```python
from build123d import *

# Parameters (mm, degrees)
SKETCH1_R           = 11.5
BOSS_EXTRUDE1_DEPTH = 4
SKETCH2_R           = 7.5
BOSS_EXTRUDE2_DEPTH = 42
CHAMFER1_SIZE       = 1
CHAMFER2_SIZE       = 0.5


with BuildPart() as part:
    # Sketch1 → Boss-Extrude1 (new body)
    with BuildSketch(Plane(origin=(0, 0, 0), x_dir=(1, 0, 0), z_dir=(0, 1, 0))):
        with Locations(Location((0, 0, 0), (0, 0, 270))):
            Circle(SKETCH1_R)
    extrude(amount=BOSS_EXTRUDE1_DEPTH)

    # Sketch2 → Boss-Extrude2 (add)
    with BuildSketch(Plane(origin=(0, 4, 0), x_dir=(1, 0, 0), z_dir=(0, 1, 0))):
        with Locations(Location((0, 0, 0), (0, 0, 90))):
            Circle(SKETCH2_R)
    extrude(amount=BOSS_EXTRUDE2_DEPTH)

    # Chamfer1
    chamfer1_edges = [part.edges().sort_by_distance(p)[0] for p in [
        (0, 46, 7.5),
    ]]
    chamfer(chamfer1_edges, length=CHAMFER1_SIZE)

    # Chamfer2
    chamfer2_edges = [part.edges().sort_by_distance(p)[0] for p in [
        (0, 0, -11.5),
        (0, 4, -11.5),
    ]]
    chamfer(chamfer2_edges, length=CHAMFER2_SIZE)


solid = part.part
```
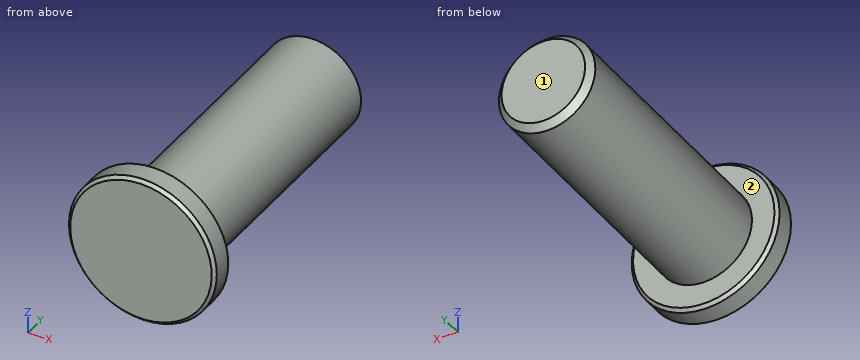
Can you work these out from the model? Positions are in its coordinate system, mm. Face numbers are marked on the shaded views. A direction names the side the tool comes from. Coordinates: 2 decimals unless noted, no trailing zeros. Write each loop counter-clockwise with the first axis right and the second up, starting at its lowest first coordinate (ties: lowest second). Pieces come first, ordered by that corner, then holes. Notation, with made-up numbers: M 72.5,52 L 83.5,52 A20 cw 83.5,57 Z; hole C -22,-19.5 d1. An arc over 180 degrees is marked long. Answer as CSV lines item,"result".
Item 1: Imagine slicing it at C-C on y = 32. List the corners of the cut face in (x, z) for me.
Geometry results:
outline,"C 0,0 d15"
Item 2: Please list where these lines run through material, in increasing order: line 1 along Y through (x, z) = (-9, 6); line 2 along Y through (x, z) = (-10.25, 5); line 3 along Z through (x, y) = (-0.5, 36.5).
Geometry results:
line 1,"y = 0 to 4"
line 2,"y = 0.4 to 3.6"
line 3,"z = -7.48 to 7.48"
Item 3: Imagine slicing it at A-A on z = 0. List the corners of the cut face in (x, y) for me, plus the area to 4 significant figures.
Geometry results:
outline,"M -11.5,0.5 L -11,0 L 11,0 L 11.5,0.5 L 11.5,3.5 L 11,4 L 7.5,4 L 7.5,45 L 6.5,46 L -6.5,46 L -7.5,45 L -7.5,4 L -11,4 L -11.5,3.5 Z"
area,"720.5 mm2"
Item 4: On a 3-axis mill with a long thin cutter (end or side, diameter ignored), from which of +Z, -Z, +X, -X, +Y, -Y can I reach the whole of each face in a straight line? I mean the marked faces 1 and 2. Say none if no direction works.
Geometry results:
face 1,"+Z, -Z, +X, -X, +Y"
face 2,"+Y"
Item 5: I'm going to push flat-ended pins straight in: P1, Ø1.5, axis at x = 8.5, z = 1.5, coming from the +Y side; P2, Ø1.5, axis at x = 7.5, z = -1, coming from the +Y side; P3, Ø12, axis at y = 30, z = 1.5, coming from the +X side. Where does each tip first touch, or does it pass through?
Geometry results:
P1,"stops at y = 4"
P2,"stops at y = 45.68"
P3,"stops at x = 7.5"
Item 6: Imagine slicing it at B-B on x = 0. List the corners of the cut face in (y, z) for me, plus the area to 4 significant figures.
Geometry results:
outline,"M 0,-11 L 0.5,-11.5 L 3.5,-11.5 L 4,-11 L 4,-7.5 L 45,-7.5 L 46,-6.5 L 46,6.5 L 45,7.5 L 4,7.5 L 4,11 L 3.5,11.5 L 0.5,11.5 L 0,11 Z"
area,"720.5 mm2"
